Build history of the part. All positions in model axes, mm. Give positions to 0.01 mm unless a question says otherwise; leave off trailing zeros. Write each loop counter-clockwise with the first axis right and the second up, starting at its lowest first coordinate (ties: lowest second). Pieces come first, ordered by that corner, then holes.
from build123d import *

# Parameters (mm, degrees)
SKETCH_1_W          = 120
SKETCH_1_H          = 25
EXTRUDE_1_DEPTH     = 1.5
SKETCH_2_R          = 6.1
CUT_EXTRUDE_1_DEPTH = 11.5


with BuildPart() as part:
    # 草图1 → 凸台-拉伸1 (new, symmetric)
    with BuildSketch(Plane.XY):
        Rectangle(SKETCH_1_W, SKETCH_1_H)
    extrude(amount=EXTRUDE_1_DEPTH, both=True)

    # 草图2 → 切除-拉伸1 (cut, symmetric)
    with BuildSketch(Plane.XY):
        Circle(SKETCH_2_R)
    extrude(amount=CUT_EXTRUDE_1_DEPTH, both=True, mode=Mode.SUBTRACT)


solid = part.part
1. Saw through at A-A on y = 0. Give the cut face in (x, z), plus the area to 3 significant figures.
2. Saw through at C-C on z = 0.2. Give the cut face in (x, y).
3. Drill centre lines: line 1 along Y through (x, z) = (0, -0.5); line 2 along X through (y, z) = (1.5, 0.4); line 3 along X through (y, z) = (-4.5, -1.15). Where is each one in solid material? Low to high.
4. Mould opens along Y. For faces 1 (the face through (-1, 12.5, 0)), 2 (the face through (60, 0, 0)), 3 (the face through (-6.094, 0.268, 0.021)) say: pulls with the +Y half, pulls with the -Y half, needs draft (parallel to the pull), parting line crosses it, or undercut.
5. Saw through at B-B on x = 4. Give the cut face in (y, z).
Outcome:
1. outline: (-60, -1.5) - (-6.1, -1.5) - (-6.1, 1.5) - (-60, 1.5) - close; (6.1, -1.5) - (60, -1.5) - (60, 1.5) - (6.1, 1.5) - close
1. area: 323 mm2
2. outline: (-60, -12.5) - (60, -12.5) - (60, 12.5) - (-60, 12.5) - close; hole circle Ø12.2 at (0, 0)
3. line 1: y = -12.5 to -6.1, 6.1 to 12.5
3. line 2: x = -60 to -5.91, 5.91 to 60
3. line 3: x = -60 to -4.12, 4.12 to 60
4. face 1: pulls with the +Y half
4. face 2: needs draft
4. face 3: undercut
5. outline: (-12.5, -1.5) - (-4.61, -1.5) - (-4.61, 1.5) - (-12.5, 1.5) - close; (4.61, -1.5) - (12.5, -1.5) - (12.5, 1.5) - (4.61, 1.5) - close
